Could you check a few things on this model? Use its own coordinates, in mm. A direction names the side the tool comes from. Round coordinates to 2 decimals unless told otherwise and drop trailing zeros. Write each loop counter-clockwise with the first axis right and the second up, starting at its lowest first coordinate (ties: lowest second). Pieces come first, ordered by that corner, then holes. Notation, with made-up numbers: (89, 40.25) - (127, 40.25) arc R11 ccw to (127, 52.25) - close; hole circle Ø2 at (39, 66.25). An arc over 180 degrees is marked (long way). Put each result on its own line as item: value.
from build123d import *

# Parameters (mm, degrees)
M5_TAPPED_HOLE1_D   = 4.2
SKETCH4_OUTSIDE_W   = 18.4
SKETCH4_OUTSIDE_H   = 18.4
SKETCH4_OUTSIDE_W_2 = 11
SKETCH4_OUTSIDE_H_2 = 11
CUT_EXTRUDE1_DEPTH  = 17.370705544


with BuildPart() as part:
    # Sketch1 → Revolve1 (revolve)
    with BuildSketch(Plane.XY):
        Polygon((0, 6), (0, 0), (14, 0), (14, 6), (11, 6), (11, 4), (3, 4), (3, 6), align=None)
    revolve(axis=Axis((14, 0, 0), (-1, 0, 0)))

    # M5 Tapped Hole1 (through all)
    with Locations(Plane.ZY):
        with Locations((0, 0)):
            Hole(M5_TAPPED_HOLE1_D / 2)

    # Sketch4 outside → Cut-Extrude1 (cut, through all)
    with BuildSketch(Plane.ZY):
        Rectangle(SKETCH4_OUTSIDE_W, SKETCH4_OUTSIDE_H)
        Rectangle(SKETCH4_OUTSIDE_W_2, SKETCH4_OUTSIDE_H_2, mode=Mode.SUBTRACT)
    extrude(amount=-CUT_EXTRUDE1_DEPTH, mode=Mode.SUBTRACT)


solid = part.part
(1) Please list where these lines run through material, in increasing order: probe 1 along X at (y, z) = (-1.75, -4.5); probe 2 along Y at (x, z) = (4.5, 0); probe 3 along Y at (x, z) = (6.25, 1). Write a range as from..to.
Values found:
probe 1: x = 0..3, 11..14
probe 2: y = -4..-2.1, 2.1..4
probe 3: y = -3.87..-1.85, 1.85..3.87
(2) If we mould it in two halves opening along Z, with no side actions, what happens to faces 3 (the face through (12, 0, -5.5)), 4 (the face through (7.098, 0.631, -2.003)), 5 (the face through (1.479, -4.265, 4.22)), 6 (the face through (1, 5.5, 0))? For each: pulls with the +Z half, pulls with the -Z half, needs draft (parallel to the pull), parting line crosses it, or undercut.
Values found:
face 3: pulls with the -Z half
face 4: undercut
face 5: pulls with the +Z half
face 6: needs draft
(3) I'm going to push flat-ended pins straight in: pin 1 (3 mm diameter, centred on x = 2.5, y = -3.5, fed in from +Z); pin 2 (2 mm diameter, centred on x = 9, z = -4, fed in from -Y). Where does each tip first touch, or does it pass through?
Values found:
pin 1: stops at z = 5.5
pin 2: stops at y = -2.65
(4) Imagine slicing it at A-A, the plane z = 0. List the corners of the cut face in (x, y) for me, then the cut area to 3 significant figures.
Values found:
outline: (0, -5.5) - (3, -5.5) - (3, -4) - (11, -4) - (11, -5.5) - (14, -5.5) - (14, -2.1) - (0, -2.1) - close; (0, 2.1) - (14, 2.1) - (14, 5.5) - (11, 5.5) - (11, 4) - (3, 4) - (3, 5.5) - (0, 5.5) - close
area: 71.2 mm^2
(5) Imagine slicing it at D-D, the plane y = -3.5. List the corners of the cut face in (x, z) for me.
Values found:
outline: (0, -4.87) - (3, -4.87) - (3, -1.94) - (11, -1.94) - (11, -4.87) - (14, -4.87) - (14, 4.87) - (11, 4.87) - (11, 1.94) - (3, 1.94) - (3, 4.87) - (0, 4.87) - close
(6) Imagine slicing it at C-C, the plane x = 11.25. List the corners of the cut face in (y, z) for me, then the cut area to 3 significant figures.
Values found:
outline: (-5.5, -2.4) arc R6 ccw to (-2.4, -5.5) - (2.4, -5.5) arc R6 ccw to (5.5, -2.4) - (5.5, 2.4) arc R6 ccw to (2.4, 5.5) - (-2.4, 5.5) arc R6 ccw to (-5.5, 2.4) - close; hole circle Ø4.2 at (0, 0)
area: 92.8 mm^2
(7) For faces 1 (the face through (14, 3, 0)), 2 (the face through (6.944, -0.867, 3.905)), which set-ups out of +Z, -Z, +X, -X, +Y, -Y let a thin tool reach every point of the face, with its end or its side?
Values found:
face 1: +Z, -Z, +X, +Y, -Y
face 2: none
